```python
from build123d import *

# Parameters (mm, degrees)
SKETCH1_R           = 3.5
BASEHEAD_DEPTH      = 4
SKETCH2_R           = 2
BASEBODY_DEPTH      = 30
HEXAGONSOCKET_DEPTH = 2
TOPFILLET_R         = 0.5
CHAMFER1_SIZE       = 0.2


with BuildPart() as part:
    # Sketch1 → BaseHead (new body)
    with BuildSketch(Plane(origin=(0, 0, 0), x_dir=(0, 0, -1), z_dir=(1, 0, 0))):
        Circle(SKETCH1_R)
    extrude(amount=BASEHEAD_DEPTH)

    # Sketch2 → BaseBody (add)
    with BuildSketch(Plane(origin=(4, 0, 0), x_dir=(0, 0, -1), z_dir=(1, 0, 0))):
        Circle(SKETCH2_R)
    extrude(amount=BASEBODY_DEPTH)

    # Sketch3 → HexagonSocket (cut)
    with BuildSketch(Plane(origin=(0, 0, 0), x_dir=(0, 0, -1), z_dir=(1, 0, 0))):
        Polygon((1.732050808, 0), (0.866025404, 1.5), (-0.866025404, 1.5), (-1.732050808, 0), (-0.866025404, -1.5), (0.866025404, -1.5), align=None)
    extrude(amount=HEXAGONSOCKET_DEPTH, mode=Mode.SUBTRACT)

    # Sketch4 → Cut-Revolve1 (revolve, cut)
    with BuildSketch(Plane(origin=(-4.19613823, 0.75, 0), x_dir=(-1, 0, 0), z_dir=(0, 0, 1)), mode=Mode.PRIVATE) as cut_revolve1_sk:
        Polygon((-6.19613823, 2.25), (-7.062163633, 0.75), (-6.19613823, 0.75), align=None)
    revolve(cut_revolve1_sk.sketch.rotate(Axis((0.838992387, 0, 0), (-1, 0, 0)), 90), axis=Axis((0.838992387, 0, 0), (-1, 0, 0)), mode=Mode.SUBTRACT)

    # TopFillet
    topfillet_edges = [part.edges().sort_by_distance(p)[0] for p in [
        (0, 0, 3.5),
    ]]
    fillet(topfillet_edges, radius=TOPFILLET_R)

    # Chamfer1
    chamfer1_edges = [part.edges().sort_by_distance(p)[0] for p in [
        (34, 0, 2),
    ]]
    chamfer(chamfer1_edges, length=CHAMFER1_SIZE)


solid = part.part
```
For this review, take the finished solid that the model builds, in its own axes (mm). A direction names the side the tool comes from. Round coordinates to 2 decimals unless told otherwise and drop trailing zeros. Write each loop counter-clockwise with the first axis right and the second up, starting at its lowest first coordinate (ties: lowest second). Pieces come first, ordered by that corner, then holes. Notation, with made-up numbers: (61.5, -32.75) -> (87.5, -32.75) arc R21 cw to (87.5, -3.75) -> close; hole circle Ø10 at (20.5, -21.5). An arc over 180 degrees is marked (long way). One line per question, with ' | ' between items. Start each with the question number.
(1) Tool access review of faces 4 (the face through (4, -2, -2)), 5 (the face through (2.226, -1.341, -3.233)), 6 (the face through (0.986, -0.76, -1.293)): name each direction out of +Z, -Z, +X, -X, +Y, -Y from which nothing blocks a thin tool from reaching the whole face with its end or side.
(2) Add section A-A, the plane x = 31.5. Write out the cut boundary in (y, z), plus the area to 3 significant figures.
(3) Mouldability with a two-part tool opening along Z and no side actions: class faces 1 (the face through (1, 1.5, 0)), 2 (the face through (0, -1.3, -1.3)), 3 (the face through (19, -2, 0)) as released by +Z, released by -Z, zero draft, split by the parting line, or undercut.
(4) For line 1 along Y through (x, z) = (9.5, -1); line 2 along X through (y, z) = (1.75, -2), list the stretches that pass through material, from the lowest coordinate up. Write a range as from..to.
(5) Insertion check: P1, Ø1.5, axis at x = 25, z = -1, coming from the +Y side; P2, Ø3, axis at x = 27.5, z = -2.5, coming from the +Y side; P3, Ø3, axis at x = 4.5, y = -2.5, coming from the +Z side. Each pin has a flat end and moves straight along its axis. Give the tip position at first contact, or say it passes through.
Answer list:
1) face 4: +X | face 5: +X, -X | face 6: -X
2) outline: circle Ø4 at (0, 0) | area: 12.6 mm²
3) face 1: undercut | face 2: zero draft | face 3: split by the parting line
4) line 1: -1.73..1.73 | line 2: 0..4
5) P1: y = 1.98 | P2: y = 1.73 | P3: z = 3.33
